Verification items for the finished model (mm, model axes). Face numbers are marked on the shaded views. Give positions to 0.01 mm unless a question says otherwise; leave off trailing zeros. Loops run counter-clockwise (first coordinate to the right, second up) from the corner with the lowest first, then second, coordinate; pieces in that order, holes last. Notation, with made-up numbers: M 4.25,-23 L 53.25,-23 A15 ccw 53.25,2 Z; hole C 23.5,-12 d11. An arc over 180 degrees is marked long. Use a Markdown table: item, result.
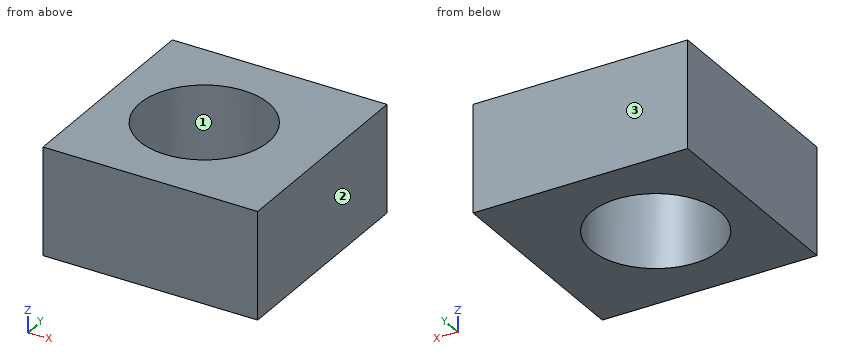
from build123d import *

# Parameters (mm, degrees)
SKETCH1_W           = 20
SKETCH1_H           = 20
SKETCH1_R           = 6
BOSS_EXTRUDE1_DEPTH = 10


with BuildPart() as part:
    # Sketch1 → Boss-Extrude1 (new body)
    with BuildSketch(Plane.XY):
        Rectangle(SKETCH1_W, SKETCH1_H)
        with Locations((-1, 0)):
            Circle(SKETCH1_R, mode=Mode.SUBTRACT)
    extrude(amount=BOSS_EXTRUDE1_DEPTH)


solid = part.part
(1) Cross-section at A-A on x = -1. Record the cut outline in (y, z).
Results below:
| item | result |
|---|---|
| outline | M -10,0 L -6,0 L -6,10 L -10,10 Z; M 6,0 L 10,0 L 10,10 L 6,10 Z |
(2) Cross-section at B-B on y = 0. Record the cut outline in (x, z), then the cut area to 3 significant figures.
Results below:
| item | result |
|---|---|
| outline | M -10,0 L -7,0 L -7,10 L -10,10 Z; M 5,0 L 10,0 L 10,10 L 5,10 Z |
| area | 80.0 mm^2 |
(3) Cross-section at C-C on z = 6. Record the cut outline in (x, y).
Results below:
| item | result |
|---|---|
| outline | M -10,-10 L 10,-10 L 10,10 L -10,10 Z; hole C -1,0 d12 |
(4) Gauge pin test, flat end, axial feed: P1, Ø8, axis at x = -1, y = 1, coming from the +Z side. Record the tip position at first contact, or that the pin passes through.
Results below:
| item | result |
|---|---|
| P1 | through |
(5) Draft check along Y on the marked faces 1, 2 and 3. Enter one of: +Y half, -Y half, draft (parallel to the pull), parting line (faces both ways), or undercut.
Results below:
| item | result |
|---|---|
| face 1 | undercut |
| face 2 | draft |
| face 3 | +Y half |
(6) Material ranges on line 1 (Y direction, x = -1, z = 4); line 2 (X direction, y = -5.5, z = 4.5); line 3 (Y direction, x = -5.25, z = 8.75), recorded low to high.
Results below:
| item | result |
|---|---|
| line 1 | -10 to -6, 6 to 10 |
| line 2 | -10 to -3.4, 1.4 to 10 |
| line 3 | -10 to -4.24, 4.24 to 10 |
